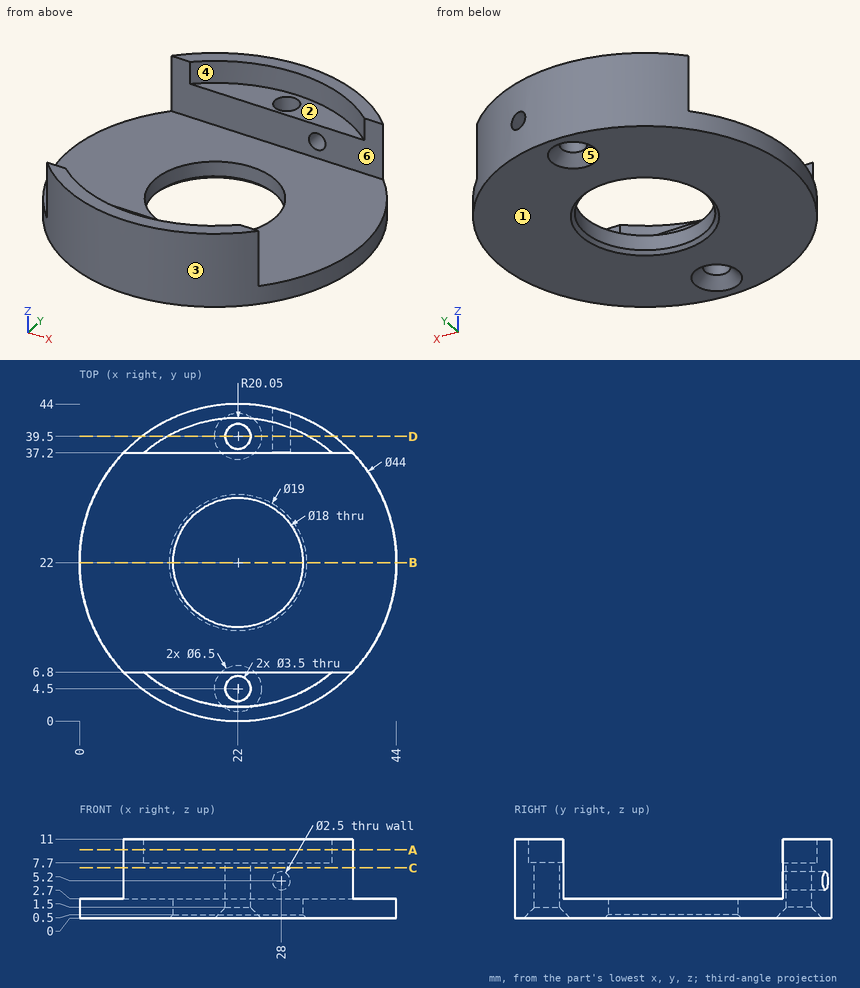
Print and shaded views of the part. All mm, measured from the part's lowest x, y and z. A direction names the side the tool comes from. Coordinates: 2 decimals unless noted, no trailing zeros. Order: outer loops, then holes, each group sorted by start corner. A loop starts at its lowest first (then second) coordinate and runs counter-clockwise, first axis right, second up.
(1) Slice it at D-D, the plane y = 39.5. Write the cut outline in (x, z).
Check sheet entries:
outline: (8.67, 0) - (18.75, 0) - (20.25, 1.5) - (20.25, 7.7) - (12.21, 7.7) - (12.21, 11) - (8.67, 11) - close; (23.75, 1.5) - (25.25, 0) - (35.33, 0) - (35.33, 11) - (31.79, 11) - (31.79, 7.7) - (23.75, 7.7) - close; hole circle Ø2.5 at (28, 5.2)
(2) Pin check, flat tips, straight feed: pin 1 Ø5 at (y, z) = (7, 3) entering from +X; pin 2 Ø2 at (x, z) = (28, 5.2) entering from +Y; pin 3 Ø4 at (x, y) = (22, 40) entering from +Z. Stop position of each tip, or through.
Check sheet entries:
pin 1: stops at x = 40.09
pin 2: stops at y = 6.8
pin 3: stops at z = 7.7
(3) Tool access for the marked faces 4, 5 and 6: list every direction of +Z, -Z, +X, -X, +Y, -Y with a clear straight run to the whole face (end or side of a thin tool).
Check sheet entries:
face 4: +Z
face 5: -Z
face 6: +Z, +X, -X
(4) Slice it at A-A, the plane z = 9.5. Write the cut outline in (x, y).
Check sheet entries:
outline: (6.1, 6.8) arc R22 ccw to (37.9, 6.8) - (35.08, 6.8) arc R20.05 cw to (8.92, 6.8) - close; (6.1, 37.2) - (8.92, 37.2) arc R20.05 cw to (35.08, 37.2) - (37.9, 37.2) arc R22 ccw to start
(5) Slice it at C-C, the plane z = 7. Write the cut outline in (x, y), and give its area (3 significant figures).
Check sheet entries:
outline: (6.1, 6.8) arc R22 ccw to (37.9, 6.8) - close; (6.1, 37.2) - (37.9, 37.2) arc R22 ccw to start; hole circle Ø3.5 at (22, 4.5); hole circle Ø3.5 at (22, 39.5)
area: 279 mm2
(6) Slice it at B-B, the plane y = 22. Write the cut outline in (x, z).
Check sheet entries:
outline: (0, 0) - (12.5, 0) - (13, 0.5) - (13, 2.7) - (0, 2.7) - close; (31, 0.5) - (31.5, 0) - (44, 0) - (44, 2.7) - (31, 2.7) - close
(7) Probe L1, parallel to Y at x = 22, z = 6; L2, parallel to Y at x = 22, z = 1.8; L3, parallel to Z at x = 18, y = 8. List the from-to ranges inside material, lowest first.
Check sheet entries:
L1: y = 0 to 2.75, 6.25 to 6.8, 37.2 to 37.75, 41.25 to 44
L2: y = 0 to 2.75, 6.25 to 13, 31 to 37.75, 41.25 to 44
L3: z = 0 to 2.7
(8) Pull direction X, two halves, no side cores. Call the marked faces 1, 2 and 3: pulls with the +X half, pulls with the -X half, needs draft (parallel to the pull), parting line crosses it, or undercut.
Check sheet entries:
face 1: needs draft
face 2: undercut
face 3: parting line crosses it
